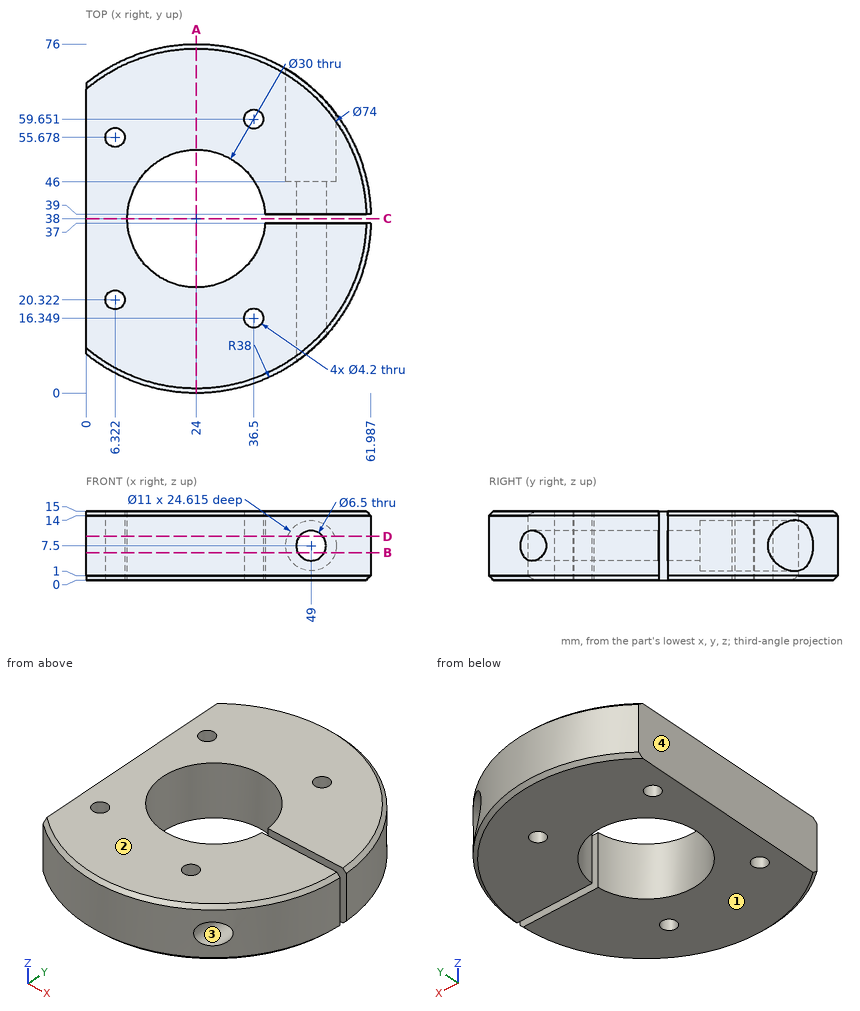
Answer from the drawing. Dimensions are ordinates in mm from the lowest x, y and z of the part. Round coordinates to 2 decimals unless told otherwise and drop trailing zeros. Loops run counter-clockwise (first coordinate to the right, second up) from the corner with the lowest first, then second, coordinate; pieces in that order, holes last.
1) A cutting plane is placed at D-D on z = 9.5. Determine the outline of the cut face in (x, y), plus the area to 3 significant figures.
Outcome:
outline: (0, 8.54) arc R38 ccw to (46.44, 7.33) - (46.44, 37) - (38.97, 37) arc R15 cw (long way) to (38.97, 39) - (46.44, 39) - (46.44, 46) - (43.88, 46) - (43.88, 70.39) arc R38 ccw to (0, 67.46) - close; (51.56, 11.84) arc R38 ccw to (61.99, 37) - (51.56, 37) - close; (51.56, 39) - (61.99, 39) arc R38 ccw to (54.12, 61.16) - (54.12, 46) - (51.56, 46) - close; hole circle Ø4.2 at (6.32, 20.32); hole circle Ø4.2 at (6.32, 55.68); hole circle Ø4.2 at (36.5, 16.35); hole circle Ø4.2 at (36.5, 59.65)
area: 2,770 mm2
2) A cutting plane is placed at C-C on y = 38. Determine the outline of the cut face in (x, z).
Outcome:
outline: (0, 0) - (9, 0) - (9, 15) - (0, 15) - close
3) Consider line 1 (Y direction, x = 6, z = 3.25) (1 decimal); line 2 (Y direction, x = 24, z = 7.5); line 3 (X direction, y = 48.5, z = 12.5) (1 decimal). Determine where each line is inside the solid, lowest interval first.
Outcome:
line 1: y = 4.5 to 18.2, 22.4 to 53.6, 57.8 to 71.5
line 2: y = 0 to 23, 53 to 76
line 3: x = 0 to 13.3, 34.7 to 46.7, 51.3 to 60.5
4) A cutting plane is placed at A-A on x = 24. Determine the outline of the cut face in (y, z), plus the area to 3 significant figures.
Outcome:
outline: (0, 1) - (1, 0) - (23, 0) - (23, 15) - (1, 15) - (0, 14) - close; (53, 0) - (75, 0) - (76, 1) - (76, 14) - (75, 15) - (53, 15) - close
area: 688 mm2
5) A cutting plane is placed at B-B on z = 6. Determine the outline of the cut face in (x, y), plus the area to 3 significant figures.
Outcome:
outline: (0, 8.54) arc R38 ccw to (46.12, 7.1) - (46.12, 37) - (38.97, 37) arc R15 cw (long way) to (38.97, 39) - (46.12, 39) - (46.12, 46) - (43.71, 46) - (43.71, 70.49) arc R38 ccw to (0, 67.46) - close; (51.88, 12.18) arc R38 ccw to (61.99, 37) - (51.88, 37) - close; (51.88, 39) - (61.99, 39) arc R38 ccw to (54.29, 60.94) - (54.29, 46) - (51.88, 46) - close; hole circle Ø4.2 at (6.32, 20.32); hole circle Ø4.2 at (6.32, 55.68); hole circle Ø4.2 at (36.5, 16.35); hole circle Ø4.2 at (36.5, 59.65)
area: 2,740 mm2
6) For a pull along Z with two mould halves and no side action, classify the marked faces 1, 2, 3 and 4 as released by +Z, released by -Z, zero draft, split by the parting line, or undercut.
Outcome:
face 1: released by -Z
face 2: released by +Z
face 3: undercut
face 4: zero draft
7) Given P1, Ø2.5, axis at x = 36.5, y = 59.65, coming from the +Z side; P2, Ø5, axis at x = 54, y = 12, coming from the -Z side; P3, Ø2, axis at x = 27, z = 10, coming from the +Y side; P4, Ø4.5, axis at x = 49, z = 9, coming from the +Y side, each flat-ended and moving along its own axis, determine where each tip first touches the part or whether it passes through.
Outcome:
P1: passes through
P2: stops at z = 0.2
P3: stops at y = 75.95
P4: stops at y = 46
